from build123d import *

# Parameters (mm, degrees)
SKETCH2_W                                           = 40
SKETCH2_H                                           = 40
BOSS_EXTRUDE1_DEPTH                                 = 4
SKETCH3_W                                           = 40
SKETCH3_H                                           = 8
BOSS_EXTRUDE2_DEPTH                                 = 25
SKETCH4_R                                           = 5.25
CUT_EXTRUDE1_DEPTH                                  = 25
CHAMFER1_SIZE                                       = 10
CBORE_FOR_M5_HEX_SOCKET_HEAD_CAP_SCREW1_D           = 5.5
CBORE_FOR_M5_HEX_SOCKET_HEAD_CAP_SCREW1_CBORE_D     = 10
CBORE_FOR_M5_HEX_SOCKET_HEAD_CAP_SCREW1_CBORE_DEPTH = 5.4
CHAMFER2_SIZE                                       = 2


with BuildPart() as part:
    # Sketch2 → Boss-Extrude1 (new body)
    with BuildSketch(Plane.XY):
        Rectangle(SKETCH2_W, SKETCH2_H)
    extrude(amount=BOSS_EXTRUDE1_DEPTH)

    # Sketch3 → Boss-Extrude2 (add)
    with BuildSketch(Plane.XY.offset(4)):
        with Locations((0, -16)):
            Rectangle(SKETCH3_W, SKETCH3_H)
    extrude(amount=BOSS_EXTRUDE2_DEPTH)

    # Sketch4 → Cut-Extrude1 (cut)
    with BuildSketch(Plane.XY.offset(4)):
        with Locations((0, 10)):
            Circle(SKETCH4_R)
    extrude(amount=-CUT_EXTRUDE1_DEPTH, mode=Mode.SUBTRACT)

    # Chamfer1
    chamfer1_edges = [part.edges().sort_by_distance(p)[0] for p in [
        (20, 20, 2),
        (-20, 20, 2),
    ]]
    chamfer(chamfer1_edges, length=CHAMFER1_SIZE)

    # CBORE for M5 Hex Socket Head Cap Screw1 (through all)
    with Locations(Plane(origin=(0, -12, 0), x_dir=(1, 0, 0), z_dir=(0, 1, 0))):
        with Locations((-14, -16.5), (14, -16.5)):
            CounterBoreHole(CBORE_FOR_M5_HEX_SOCKET_HEAD_CAP_SCREW1_D / 2, CBORE_FOR_M5_HEX_SOCKET_HEAD_CAP_SCREW1_CBORE_D / 2, CBORE_FOR_M5_HEX_SOCKET_HEAD_CAP_SCREW1_CBORE_DEPTH)

    # Chamfer2
    chamfer2_edges = [part.edges().sort_by_distance(p)[0] for p in [
        (20, -16, 29),
        (-20, -16, 29),
    ]]
    chamfer(chamfer2_edges, length=CHAMFER2_SIZE)


solid = part.part
Can you work these out from the model? Positions are in its coordinate system, mm. A direction names the side the tool comes from. Round coordinates to 2 decimals unless told otherwise and drop trailing zeros. Loops run counter-clockwise (first coordinate to the right, second up) from the corner with the lowest first, then second, coordinate; pieces in that order, holes last. Notation, with made-up numbers: (-39.5, 75) - (-8.5, 75) arc R28 ccw to (-8.5, 109) - close; hole circle Ø3 at (70, 58.25). An arc over 180 degrees is marked (long way). Write item = value, one per line. Start each with the question number.
(1) For faces 1 (the face through (16, -17.4, 19)), 2 (the face through (-11.973, -18.718, 14.641)), 3 (the face through (0, -12, 16)), which set-ups out of +Z, -Z, +X, -X, +Y, -Y let a thin tool reach every point of the face, with its end or its side?
(2) If we section it at D-D (x = 0): Please give me the cut outline in (y, z), and give its area (3 significant figures).
(3) If we section it at A-A (y = -16): Please give me the cut outline in (x, z).
(4) If I drill on probe 1 along X at (y, z) = (-18.7, 16.5); probe 2 along X at (y, z) = (-14, 16.5); probe 3 along Z at (x, y) = (-14, -13), over which ranges is the centre line in solid material (lowest first)? Write a range as [from, to].
(5) If we section it at C-C (z = 16.5): Please give me the cut outline in (x, y).
(6) For P1, Ø8, axis at x = 14, z = 18, coming from the +Y side; P2, Ø3, axis at x = -15.5, z = 15, coming from the +Y side; P3, Ø1, axis at x = 15.5, y = 9.5, coming from the +Z side, each with a flat end and sliding along its axis, tell me the tip position at first contact or that it passes through.
(7) If we mould it in two halves opening along Z, with no side actions, what happens to faces 4 (the face through (-20, -13, 11)), 5 (the face through (0, 0, 0)), 6 (the face through (16.307, -14.662, 20.936)), 7 (the face through (16.747, -18.718, 16.379))? For each: released by +Z, released by -Z, zero draft, split by the parting line, or undercut.
(8) If we section it at B-B (x = 14): Please give me the cut outline in (y, z).
Ans:
q1.face_1 = +Y
q1.face_2 = +Y, -Y
q1.face_3 = +Z, +X, -X, +Y
q2.outline = (-20, 0) - (4.75, 0) - (4.75, 4) - (-12, 4) - (-12, 29) - (-20, 29) - close; (15.25, 0) - (20, 0) - (20, 4) - (15.25, 4) - close
q2.area = 318 mm²
q3.outline = (-20, 0) - (20, 0) - (20, 27) - (18, 29) - (-18, 29) - (-20, 27) - close; hole circle Ø10 at (-14, 16.5); hole circle Ø10 at (14, 16.5)
q4.probe_1 = [-20, -16.75], [-11.25, 11.25], [16.75, 20]
q4.probe_2 = [-20, -19], [-9, 9], [19, 20]
q4.probe_3 = [0, 11.5], [21.5, 29]
q5.outline = (-20, -20) - (-16.75, -20) - (-16.75, -17.4) - (-19, -17.4) - (-19, -12) - (-20, -12) - close; (-11.25, -20) - (11.25, -20) - (11.25, -17.4) - (9, -17.4) - (9, -12) - (-9, -12) - (-9, -17.4) - (-11.25, -17.4) - close; (16.75, -20) - (20, -20) - (20, -12) - (19, -12) - (19, -17.4) - (16.75, -17.4) - close
q6.P1 = -12
q6.P2 = -17.4
q6.P3 = 4
q7.face_4 = zero draft
q7.face_5 = released by -Z
q7.face_6 = undercut
q7.face_7 = undercut
q8.outline = (-20, 0) - (16, 0) - (16, 4) - (-12, 4) - (-12, 11.5) - (-17.4, 11.5) - (-17.4, 13.75) - (-20, 13.75) - close; (-20, 19.25) - (-17.4, 19.25) - (-17.4, 21.5) - (-12, 21.5) - (-12, 29) - (-20, 29) - close
